```python
from build123d import *

# Parameters (mm, degrees)
EXTRUDE_1_DEPTH  = 3
SKETCH_2_R       = 23
SKETCH_2_R_2     = 20
EXTRUDE_2_DEPTH  = 100
SKETCH_4_W       = 3
SKETCH_4_H       = 50
EXTRUDE_3_DEPTH  = 715
SKETCH_7_W       = 506.314990664
SKETCH_7_H       = 3
EXTRUDE_8_DEPTH  = 30
SKETCH_8_W       = 3
SKETCH_8_H       = 35
SKETCH_8_H_2     = 100
EXTRUDE_9_DEPTH  = 30
SKETCH_9_W       = 3
SKETCH_9_H       = 50
EXTRUDE_10_DEPTH = 187


with BuildPart() as part:
    # Sketch 1 → Extrude 1 (new body)
    with BuildSketch(Plane(origin=(0, 0, 0), x_dir=(1, 0, 0), z_dir=(0, 1, 0))):
        Polygon((357.5, -60), (152.5, -60), (152.5, 0), (0, 0), (0, 190), (715, 190), (715, 0), (562.5, 0), (562.5, -60), align=None)
    extrude(amount=EXTRUDE_1_DEPTH)

    # Sketch 2 → Extrude 2 (add)
    # profile 1 of 2: a face of its own
    with BuildSketch(Plane(origin=(0, 3, 0), x_dir=(1, 0, 0), z_dir=(0, 1, 0))):
        with Locations(Location((80, 155, 0), (0, 0, 90))):
            Circle(SKETCH_2_R)
        with Locations(Location((80, 155, 0), (0, 0, 270))):
            Circle(SKETCH_2_R_2, mode=Mode.SUBTRACT)
    # profile 2 of 2: a face of its own
    with BuildSketch(Plane(origin=(0, 3, 0), x_dir=(1, 0, 0), z_dir=(0, 1, 0))):
        with Locations(Location((635, 155, 0), (0, 0, 90))):
            Circle(SKETCH_2_R)
        with Locations(Location((635, 155, 0), (0, 0, 270))):
            Circle(SKETCH_2_R_2, mode=Mode.SUBTRACT)
    extrude(amount=EXTRUDE_2_DEPTH)

    # Sketch 7 → Extrude 8 (add)
    with BuildSketch(Plane(origin=(0, 3, 0), x_dir=(1, 0, 0), z_dir=(0, 1, 0))):
        with Locations((357.381396842, 153.5)):
            Rectangle(SKETCH_7_W, SKETCH_7_H)
    extrude(amount=EXTRUDE_8_DEPTH)

    # Sketch 8 → Extrude 9 (add)
    with BuildSketch(Plane(origin=(0, 3, 0), x_dir=(1, 0, 0), z_dir=(0, 1, 0))):
        with Locations((251.5, 172.5)):
            Rectangle(SKETCH_8_W, SKETCH_8_H)
        with Locations((251.5, 102)):
            Rectangle(SKETCH_8_W, SKETCH_8_H_2)
        with Locations((463.5, 102)):
            Rectangle(SKETCH_8_W, SKETCH_8_H_2)
        with Locations((463.5, 172.5)):
            Rectangle(SKETCH_8_W, SKETCH_8_H)
    extrude(amount=EXTRUDE_9_DEPTH)



with BuildPart() as body_2:
    # Sketch 4 → Extrude 3 (new body)
    with BuildSketch(Plane(origin=(715, 0, 0), x_dir=(0, 0, -1), z_dir=(1, 0, 0))):
        with Locations((188.5, -25)):
            Rectangle(SKETCH_4_W, SKETCH_4_H)
    extrude(amount=-EXTRUDE_3_DEPTH)


with BuildPart() as part_1:
    add(part.part)

    add(body_2.part)  # Extrude 10 merges body 2
    # Sketch 9 → Extrude 10 (add)
    with BuildSketch(Plane.XY):
        with Locations((713.5, -25)):
            Rectangle(SKETCH_9_W, SKETCH_9_H)
        with Locations((1.5, -25)):
            Rectangle(SKETCH_9_W, SKETCH_9_H)
    extrude(amount=-EXTRUDE_10_DEPTH)


solid = part_1.part
```
Can you work these out from the model? Positions are in its coordinate system, mm. A direction names the side the tool comes from. Round coordinates to 2 decimals unless told otherwise and drop trailing zeros. Loops run counter-clockwise (first coordinate to the right, second up) from the corner with the lowest first, then second, coordinate; pieces in that order, holes last. Notation, with made-up numbers: M -27,-40 L -11,-40 A36 ccw -11,-2 Z; hole C 7,-38.5 d9. An arc over 180 degrees is marked long. Answer as a JSON object with one key per item and string values. Group by question number.
Q1. We'd pull the mould along Z, two halves only. Please class faces 4 (the flat face through (253, 18, -101)), 5 (the flat face through (635, 3, -155)), 6 (the cylindrical face through (94, 52.3, -136.75)), 7 (the flat face through (176, 18, -155)): +Z half, -Z half, draft (parallel to the pull), parting line (faces both ways), or undercut.
Q2. Will these pins go through, and if not, where does the flat tip stop? pin 1 (1.5 mm diameter, centred on y = 15, z = -153, fed in from -X); pin 2 (12 mm diameter, centred on x = 638.5, z = -154, fed in from +Y); pin 3 (2 mm diameter, centred on y = 5.5, z = -149.5, fed in from +X).
Q3. Imagine slicing it at B-B, the plane x = 593. Please give me the cut outline in (y, z).
Q4. On a 3-axis mill with a long thin cutter (end or side, diameter ignored), from which of +Z, -Z, +X, -X, +Y, -Y can I reach the whole of each face in a straight line? I mean faces 1 (the cylindrical face through (68, 52, -171)), 2 (the flat face through (465, 18, -172)), 3 (the flat face through (3, -25, -92)). Say none if no direction works.
Q5. Please list where these lines run through material, in increasing order: L1, parallel to X at y = 43.5, z = -155; L2, parallel to X at y = -27.5, z = -72.5; L3, parallel to X at y = 64, z = -141.5.
Q6. Imagine slicing it at C-C, the plane z = -23. Please give me the cut outline in (x, y), then the cut area to 4 significant figures.
Q7. Imagine slicing it at A-A, the plane y = 48. Please give me the cut outline in (x, z), then the cut area to 3 significant figures.
Q8. Imagine slicing it at D-D, the plane y = -24. Please give me the cut outline in (x, z), then the cut area to 3 significant figures.
Findings:
{
 "1": {"face 4": "draft", "face 5": "undercut", "face 6": "parting line", "face 7": "-Z half"},
 "2": {"pin 1": "stops at x = 57.03", "pin 2": "stops at y = 3", "pin 3": "stops at x = 657.56"},
 "3": {"outline": "M -50,-190 L 3,-190 L 3,-155 L 33,-155 L 33,-152 L 3,-152 L 3,0 L 0,0 L 0,-187 L -50,-187 Z"},
 "4": {"face 1": "+Y", "face 2": "-Z, +Y", "face 3": "+Z, -Y"},
 "5": {"L1": "x = 57 to 60, 100 to 103, 612 to 615, 655 to 658", "L2": "x = 0 to 3, 712 to 715", "L3": "x = 61.38 to 65.24, 94.76 to 98.62, 616.38 to 620.24, 649.76 to 653.62"},
 "6": {"outline": "M 0,-50 L 3,-50 L 3,0 L 712,0 L 712,-50 L 715,-50 L 715,3 L 0,3 Z", "area": "2,445 mm2"},
 "7": {"outline": "C 80,-155 d46; C 635,-155 d46; hole C 80,-155 d40; hole C 635,-155 d40", "area": "811 mm2"},
 "8": {"outline": "M 0,-190 L 715,-190 L 715,0 L 712,0 L 712,-187 L 3,-187 L 3,0 L 0,0 Z", "area": "3,270 mm2"}
}
